Design review of the part built by this model. Coordinates are the model's own, in mm. A direction names the side the tool comes from. Give positions to 0.01 mm unless a question says otherwise; leave off trailing zeros. Loops run counter-clockwise (first coordinate to the right, second up) from the corner with the lowest first, then second, coordinate; pieces in that order, holes last. Notation, with made-up numbers: (64, -1.75) - (121, -1.75) arc R26 ccw to (121, 28.25) - close; hole circle Ø4 at (50.5, -7.5). An arc over 180 degrees is marked (long way). Write each question's results on one line, items separated by ' | '.
from build123d import *

# Parameters (mm, degrees)
HUB_RING_SKETCH_R     = 32.5
HUB_RING_SKETCH_R_2   = 22.5
HUB_RING_65X_45_DEPTH = 20
FORK_ARM_DEPTH        = 20
REAR_TAB_DEPTH        = 20


with BuildPart() as part:
    # Hub Ring Sketch → Hub Ring Ø65xØ45 (new, symmetric)
    with BuildSketch(Plane(origin=(0, 0, 0), x_dir=(1, 0, 0), z_dir=(0, 1, 0))):
        with Locations(Location((0, 0, 0), (0, 0, 270))):
            Circle(HUB_RING_SKETCH_R)
        with Locations(Location((0, 0, 0), (0, 0, 270))):
            Circle(HUB_RING_SKETCH_R_2, mode=Mode.SUBTRACT)
    extrude(amount=HUB_RING_65X_45_DEPTH, both=True)

    # Fork Arm Sketch → Fork Arm (add)
    with BuildSketch(Plane(origin=(0, 0, 0), x_dir=(1, 0, 0), z_dir=(0, 1, 0))):
        with BuildLine():
            Line((95.760171689, 18.152180955), (4.941115981, 32.122194397))
            ThreePointArc((4.941115981, 32.122194397), (32.5, 0), (4.941115981, -32.122194397))
            Line((4.941115981, -32.122194397), (95.760171689, -18.152180955))
            ThreePointArc((95.760171689, -18.152180955), (98.794789747, -16.466003095), (100, -13.210304894))
            Line((100, -13.210304894), (100, -9))
            Line((100, -9), (68, -9))
            ThreePointArc((68, -9), (59, 0), (68, 9))
            Line((68, 9), (100, 9))
            Line((100, 9), (100, 13.210304894))
            ThreePointArc((100, 13.210304894), (98.794789747, 16.466003095), (95.760171689, 18.152180955))
        make_face()
    extrude(amount=-FORK_ARM_DEPTH)

    # Rear Tab Sketch → Rear Tab (add)
    with BuildSketch(Plane(origin=(0, 0, 0), x_dir=(1, 0, 0), z_dir=(0, 1, 0))):
        with BuildLine():
            Line((-28.831406487, 15), (-55, 15))
            Line((-55, 15), (-55, -15))
            Line((-55, -15), (-28.831406487, -15))
            ThreePointArc((-28.831406487, -15), (-32.5, 0), (-28.831406487, 15))
        make_face()
    extrude(amount=-REAR_TAB_DEPTH)


solid = part.part
(1) Tool access review of faces 4 (the flat face through (22, 20, 7)), 5 (the flat face through (-42, -10, -15)), 6 (the flat face through (84, -10, 9)), 7 (the cylindrical face through (-19.78, 4.72, -25.79)), 8 (the flat face through (-42, -10, 15)): name each direction out of +Z, -Z, +X, -X, +Y, -Y from which nothing blocks a thin tool from reaching the whole face with its end or side.
Answers below:
face 4: +Z, -Z, +X, -X, +Y | face 5: -Z, -X, +Y, -Y | face 6: +X, +Y, -Y | face 7: +Y | face 8: +Z, -X, +Y, -Y
(2) Insertion check: P1, Ø22, axis at x = 87, y = -14.5, coming from the +Z side; P2, Ø1.5, axis at x = 16, y = 1, coming from the -Z side; P3, Ø3, axis at x = 24, y = -15, coming from the +Z side. Each pin has a flat end and moves straight along its axis. Give the tip position at first contact, or say it passes through.
Answers below:
P1: z = 21.19 | P2: z = -28.7 | P3: z = 29.42
(3) Take a section at D-D on y = 10. Give the boundary of the cut face in (x, z).
Answers below:
outline: circle Ø65 at (0, 0); hole circle Ø45 at (0, 0)
(4) Wall thickness on line 1 along X through (y, z) = (5.5, 1); line 2 along X through (y, z) = (-3.5, 0); line 3 along Y through (x, z) = (-35, -10.5): over which ranges is each line inside the solid? List them lowest first. Write a range as from..to.
Answers below:
line 1: -32.48..-22.48, 22.48..32.48 | line 2: -55..-22.5, 22.5..59 | line 3: -20..0
(5) Draft analysis for pull direction Z (two halves, no side actions). For faces 1 (the flat face through (49.715, -9.86, 25.235)), 2 (the flat face through (84, -10, -9)), 3 (the flat face through (50.99, -9.86, -25.04)), state which applies: pulls with the +Z half, pulls with the -Z half, needs draft (parallel to the pull), parting line crosses it, or undercut.
Answers below:
face 1: pulls with the +Z half | face 2: undercut | face 3: pulls with the -Z half
(6) Take a section at A-A on z = 0. Give the boundary of the cut face in (x, y).
Answers below:
outline: (-55, -20) - (-22.5, -20) - (-22.5, 20) - (-32.5, 20) - (-32.5, 0) - (-55, 0) - close; (22.5, -20) - (59, -20) - (59, 0) - (32.5, 0) - (32.5, 20) - (22.5, 20) - close
(7) Take a section at C-C on y = -10. Give the boundary of the cut face in (x, z).
Answers below:
outline: (-55, -15) - (-28.83, -15) arc R32.5 ccw to (4.94, -32.12) - (95.76, -18.15) arc R5 ccw to (100, -13.21) - (100, -9) - (68, -9) arc R9 cw to (68, 9) - (100, 9) - (100, 13.21) arc R5 ccw to (95.76, 18.15) - (4.94, 32.12) arc R32.5 ccw to (-28.83, 15) - (-55, 15) - close; hole circle Ø45 at (0, 0)
(8) Take a section at B-B on x = 0. Give the boundary of the cut face in (y, z).
Answers below:
outline: (-20, -32.5) - (20, -32.5) - (20, -22.5) - (-20, -22.5) - close; (-20, 22.5) - (20, 22.5) - (20, 32.5) - (-20, 32.5) - close
